```python
from build123d import *

# Parameters (mm, degrees)
SKETCH1_R           = 135
BOSS_EXTRUDE2_DEPTH = 20
SKETCH5_W           = 270
SKETCH5_H           = 200
CUT_EXTRUDE1_DEPTH  = 20
SKETCH6_W           = 245
SKETCH6_H           = 100
SKETCH6_W_2         = 135
BOSS_EXTRUDE3_DEPTH = 20


with BuildPart() as part:
    # Sketch1 → Boss-Extrude2 (new body)
    with BuildSketch(Plane.XY):
        with BuildLine():
            Line((-135, 475), (-135, 94.868329805))
            ThreePointArc((-135, 94.868329805), (-165, 0), (-135, -94.868329805))
            Line((-135, -94.868329805), (-135, -475))
            Line((-135, -475), (135, -475))
            Line((135, -475), (135, -94.868329805))
            ThreePointArc((135, -94.868329805), (165, 0), (135, 94.868329805))
            Line((135, 94.868329805), (135, 475))
            Line((135, 475), (-135, 475))
        make_face()
        Circle(SKETCH1_R, mode=Mode.SUBTRACT)
    extrude(amount=BOSS_EXTRUDE2_DEPTH)

    # Sketch5 → Cut-Extrude1 (cut)
    with BuildSketch(Plane.XY.offset(20)):
        with Locations((0, -375)):
            Rectangle(SKETCH5_W, SKETCH5_H)
    extrude(amount=-CUT_EXTRUDE1_DEPTH, mode=Mode.SUBTRACT)

    # Sketch6 → Boss-Extrude3 (add)
    with BuildSketch(Plane(origin=(0, 0, 0), x_dir=(-1, 0, 0), z_dir=(0, 0, -1))):
        with Locations((-257.5, 425)):
            Rectangle(SKETCH6_W, SKETCH6_H)
        with Locations((202.5, 425)):
            Rectangle(SKETCH6_W_2, SKETCH6_H)
    extrude(amount=-BOSS_EXTRUDE3_DEPTH)


solid = part.part
```
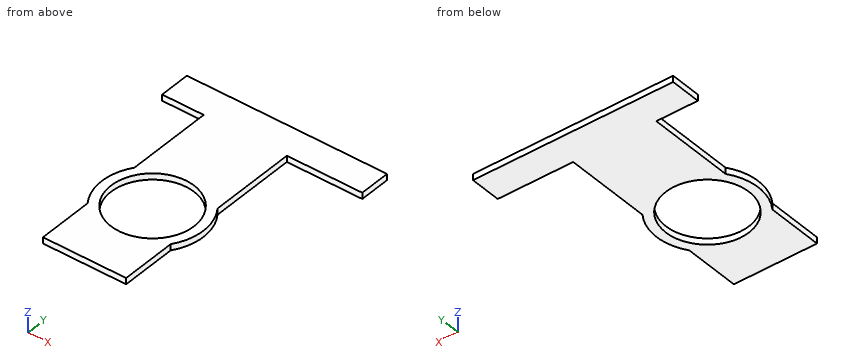
For this review, take the finished solid that the model builds, in its own axes (mm). Give positions to 0.01 mm unless a question says otherwise; leave off trailing zeros. Loops run counter-clockwise (first coordinate to the right, second up) from the corner with the lowest first, then second, coordinate; pieces in that order, holes last. Notation, with made-up numbers: M 69.5,56 L 119.5,56 A37 cw 119.5,93 Z; hole C 68,60 d4. An arc over 180 degrees is marked long. One line per item, written item: value. Start each with the question number.
Q1. Add section B-B (y = 0). Give the boundary of the cut face in (x, z).
Q2. Add section A-A (x = 0). Give the boundary of the cut face in (y, z).
Q3. Add section D-D (x = 333). Give the boundary of the cut face in (y, z).
Q4. Clearance check with flat-ended pins moving along their axes: pin 1 Ø3 at (y, z) = (225.5, 14.5) entering from +X; pin 2 Ø6 at (x, z) = (306, 8) entering from -Y; pin 3 Ø3 at (y, z) = (-48, 14.5) entering from +X. State where each tip first meets the part, or that it passes through.
Q5. Add section C-C (z = 5.5). Give the boundary of the cut face in (x, y).
Q6. For L1, parallel to Y at x = 0, z = 10.75; L2, parallel to X at y = 247.5, z = 17.5; L3, parallel to Y at x = -28, z = 2, list the stretches that pass through material, from the lowest coordinate up.
Reply:
1. outline: M -165,0 L -135,0 L -135,20 L -165,20 Z; M 135,0 L 165,0 L 165,20 L 135,20 Z
2. outline: M -275,0 L -135,0 L -135,20 L -275,20 Z; M 135,0 L 475,0 L 475,20 L 135,20 Z
3. outline: M 375,0 L 475,0 L 475,20 L 375,20 Z
4. pin 1: x = 135
4. pin 2: y = 375
4. pin 3: x = 158.31
5. outline: M -270,375 L -135,375 L -135,94.87 A165 ccw -135,-94.87 L -135,-275 L 135,-275 L 135,-94.87 A165 ccw 135,94.87 L 135,375 L 380,375 L 380,475 L -270,475 Z; hole C 0,0 d270
6. L1: -275 to -135, 135 to 475
6. L2: -135 to 135
6. L3: -275 to -132.06, 132.06 to 475
